```python
from build123d import *

# Parameters (mm, degrees)
EXTRUDE_1_DEPTH     = 5
SKETCH_2_W          = 21.5
SKETCH_2_H          = 41.5
CUT_EXTRUDE_1_DEPTH = 5
FILLET_1_R          = 10


with BuildPart() as part:
    # 草图1 → 凸台-拉伸1 (new body)
    with BuildSketch(Plane.XY):
        Polygon((-27.85, 37.5), (-27.85, 15), (-32.85, 15), (-32.85, 5), (-27.85, 5), (-27.85, -5), (-32.85, -5), (-32.85, -15), (-27.85, -15), (-27.85, -37.5), (27.85, -37.5), (27.85, -15), (32.85, -15), (32.85, -5), (27.85, -5), (27.85, 5), (32.85, 5), (32.85, 15), (27.85, 15), (27.85, 37.5), align=None)
    extrude(amount=EXTRUDE_1_DEPTH)

    # 草图2 → 切除-拉伸1 (cut)
    with BuildSketch(Plane.XY.offset(5)):
        Rectangle(SKETCH_2_W, SKETCH_2_H)
    extrude(amount=-CUT_EXTRUDE_1_DEPTH, mode=Mode.SUBTRACT)

    # 圆角1
    fillet_1_edges = [part.edges().sort_by_distance(p)[0] for p in [
        (27.85, -37.5, 2.5),
        (-27.85, -37.5, 2.5),
        (-27.85, 37.5, 2.5),
        (27.85, 37.5, 2.5),
    ]]
    fillet(fillet_1_edges, radius=FILLET_1_R)


solid = part.part
```
The listing builds one solid part. Answer for the finished solid, in the listing's coordinates (mm). A direction names the side the tool comes from. Round coordinates to 2 decimals unless told otherwise and drop trailing zeros. Write each loop counter-clockwise with the first axis right and the second up, starting at its lowest first coordinate (ties: lowest second). Pieces come first, ordered by that corner, then holes. Notation, with made-up numbers: (-19, -9) -> (13, -9) arc R12 cw to (13, 2) -> close; hole circle Ø4 at (76, 36.5). An arc over 180 degrees is marked (long way). Use CSV: the item, a comma, the result in double quotes. Start each with the question number.
(1) Section A-A on x = 9.5 is taken. Give the vertices of the cut face in (y, z).
(2) The mould has two halves that part along X. Classify faces 6 (the face through (-10.75, 0, 3)), 7 (the face through (24.84, 34.65, 2.54)), 8 (the face through (-27.85, 0, 2)), 9 (the face through (-30, -15, 2)): released by +X, released by -X, zero draft, split by the parting line, or undercut.
(3) Section B-B on y = 13 is taken. Give the vertices of the cut face in (x, z), then the cut area to 3 significant figures.
(4) Each of these flat-tipped pins is pushed along its axis until it touches: pin 1 (1.5 mm diameter, centred on y = 1.5, z = 3, fed in from +X); pin 2 (1.5 mm diameter, centred on x = 30, z = 1.5, fed in from -Y); pin 3 (2.5 mm diameter, centred on x = -31, z = 3, fed in from +Y). Where does it stop, or does it pass through?
(5) Consider L1, parallel to X at y = 13, z = 0.65; L2, parallel to X at y = -17, z = 2.65; L3, parallel to Y at x = -6.5, z = 4.4. Determine where each line is inside the solid, lowest interval first. Write a range as from..to.
(6) Section D-D on y = 26 is taken. Give the vertices of the cut face in (x, z).
(7) Which of the six approach directions +Z, -Z, +X, -X, +Y, -Y give full straight-line access (tool end or side, diameter ignored) to faces 1 (the face through (0, 20.75, 3)), 2 (the face through (30, 5, 2)), 3 (the face through (-27.85, 21, 2)), 4 (the face through (-27.85, -21, 2)), 5 (the face through (30, 15, 2))?
(8) Section C-C on z = 0.85 is taken. Give the vertices of the cut face in (x, y), then the cut area to 3 significant figures.
A:
1,outline,"(-37.5, 0) -> (-20.75, 0) -> (-20.75, 5) -> (-37.5, 5) -> close; (20.75, 0) -> (37.5, 0) -> (37.5, 5) -> (20.75, 5) -> close"
2,face 6,"undercut"
2,face 7,"released by +X"
2,face 8,"released by -X"
2,face 9,"zero draft"
3,outline,"(-32.85, 0) -> (-10.75, 0) -> (-10.75, 5) -> (-32.85, 5) -> close; (10.75, 0) -> (32.85, 0) -> (32.85, 5) -> (10.75, 5) -> close"
3,area,"221 mm²"
4,pin 1,"stops at x = 27.85"
4,pin 2,"stops at y = -15"
4,pin 3,"stops at y = 15"
5,L1,"x = -32.85..-10.75, 10.75..32.85"
5,L2,"x = -27.85..-10.75, 10.75..27.85"
5,L3,"y = -37.5..-20.75, 20.75..37.5"
6,outline,"(-27.85, 0) -> (27.85, 0) -> (27.85, 5) -> (-27.85, 5) -> close"
7,face 1,"+Z, -Z"
7,face 2,"+Z, -Z, +X"
7,face 3,"+Z, -Z, -X, +Y"
7,face 4,"+Z, -Z, -X, -Y"
7,face 5,"+Z, -Z, +X, +Y"
8,outline,"(-32.85, -15) -> (-27.85, -15) -> (-27.85, -27.5) arc R10 ccw to (-17.85, -37.5) -> (17.85, -37.5) arc R10 ccw to (27.85, -27.5) -> (27.85, -15) -> (32.85, -15) -> (32.85, -5) -> (27.85, -5) -> (27.85, 5) -> (32.85, 5) -> (32.85, 15) -> (27.85, 15) -> (27.85, 27.5) arc R10 ccw to (17.85, 37.5) -> (-17.85, 37.5) arc R10 ccw to (-27.85, 27.5) -> (-27.85, 15) -> (-32.85, 15) -> (-32.85, 5) -> (-27.85, 5) -> (-27.85, -5) -> (-32.85, -5) -> close; hole (-10.75, -20.75) -> (10.75, -20.75) -> (10.75, 20.75) -> (-10.75, 20.75) -> close"
8,area,"3,400 mm²"
